```python
from build123d import *


with BuildPart() as part:
    # 草图1 → 旋转1 (revolve)
    with BuildSketch(Plane.XY, mode=Mode.PRIVATE) as revolve_1_sk:
        Polygon((11.5, 2), (9.5, 2), (9.5, 3), (10, 3), (10, 36), (9.5, 36), (9.5, 37.25), (10, 37.25), (10, 39), (9, 40), (0, 40), (0, 0), (11.5, 0), (12, 0.5), (12, 1.5), align=None)
    revolve(revolve_1_sk.sketch.rotate(Axis((0, -1.467272455, 0), (0, 1, 0)), 90), axis=Axis((0, -1.467272455, 0), (0, 1, 0)))


solid = part.part
```
Geometry: final body of the model. Coordinates: model frame, mm. A direction names the side the tool comes from. Round coordinates to 2 decimals unless told otherwise and drop trailing zeros. Order: outer loops, then holes, each group sorted by start corner. A loop starts at its lowest first (then second) coordinate and runs counter-clockwise, first axis right, second up. Notation, with made-up numbers: (50, -35.75) -> (86, -35.75) arc R21 ccw to (86, -20.75) -> close; hole circle Ø4 at (72.5, -7.5). An arc over 180 degrees is marked (long way). Write each question's results on one line, items separated by ' | '.
Q1. Pull-direction query (Y, two-part tool) for faces 1 (the face through (0, 40, 0)), 2 (the face through (4, 36, -9)), 3 (the face through (0, 20, 10)), 4 (the face through (0, 0, 0)); classes: released by +Y, released by -Y, zero draft, split by the parting line, or undercut.
Response values:
face 1: released by +Y | face 2: undercut | face 3: zero draft | face 4: released by -Y
Q2. Section query B-B (x = 0). Output: boundary loops of the cut face in (y, z), and give its area (3 significant figures).
Response values:
outline: (0, -11.5) -> (0.5, -12) -> (1.5, -12) -> (2, -11.5) -> (2, -9.5) -> (3, -9.5) -> (3, -10) -> (36, -10) -> (36, -9.5) -> (37.25, -9.5) -> (37.25, -10) -> (39, -10) -> (40, -9) -> (40, 9) -> (39, 10) -> (37.25, 10) -> (37.25, 9.5) -> (36, 9.5) -> (36, 10) -> (3, 10) -> (3, 9.5) -> (2, 9.5) -> (2, 11.5) -> (1.5, 12) -> (0.5, 12) -> (0, 11.5) -> close | area: 804 mm²
Q3. Access query for faces 5 (the face through (-3.604, 1.007, -11.446)), 6 (the face through (4, 37.25, 9)), 7 (the face through (0, 38, 10)). Directions: +Z, -Z, +X, -X, +Y, -Y. A direction counts if a zero-diameter tool reaches every point of the face in a straight line with its end or side. Return the directions, or none.
Response values:
face 5: +Y, -Y | face 6: none | face 7: +Y
Q4. Section query C-C (y = 13). Output: boundary loops of the cut face in (x, z), and give its area (3 significant figures).
Response values:
outline: circle Ø20 at (0, 0) | area: 314 mm²
Q5. Ray query, line 1 along Y through (x, z) = (-2.5, -10.75); line 2 along Y through (x, z) = (-2, -9.75); line 3 along Y through (x, z) = (10.5, 5). Return the intervals inside material, ascending.
Response values:
line 1: 0 to 2 | line 2: 0 to 2, 3 to 36, 37.25 to 39.05 | line 3: 0.13 to 1.87
Q6. Section query A-A (z = 0). Output: boundary loops of the cut face in (x, y).
Response values:
outline: (-12, 0.5) -> (-11.5, 0) -> (11.5, 0) -> (12, 0.5) -> (12, 1.5) -> (11.5, 2) -> (9.5, 2) -> (9.5, 3) -> (10, 3) -> (10, 36) -> (9.5, 36) -> (9.5, 37.25) -> (10, 37.25) -> (10, 39) -> (9, 40) -> (-9, 40) -> (-10, 39) -> (-10, 37.25) -> (-9.5, 37.25) -> (-9.5, 36) -> (-10, 36) -> (-10, 3) -> (-9.5, 3) -> (-9.5, 2) -> (-11.5, 2) -> (-12, 1.5) -> close
Q7. Pin query (flat end, axial travel): pin 1 Ø1 at (y, z) = (22.5, 8) entering from -X; pin 2 Ø5 at (y, z) = (14, 3.5) entering from -X; pin 3 Ø5 at (x, y) = (7, 8) entering from -Z. Return the tip coordinate at first contact, or that it passes through.
Response values:
pin 1: x = -6.61 | pin 2: x = -9.95 | pin 3: z = -8.93
